Could you check a few things on this model? Use its own coordinates, in mm. Round coordinates to 2 decimals unless told otherwise and drop trailing zeros. Write each loop counter-clockwise with the first axis right and the second up, starting at its lowest first coordinate (ties: lowest second). Pieces come first, ordered by that corner, then holes. Notation, with made-up numbers: (75, -17) - (82, -17) arc R15 ccw to (82, 11) - close; hole circle Ø10 at (-33.5, 74). An arc over 180 degrees is marked (long way). Write each question's results on one line, items separated by ' | '. Start each with the question number.
(1) For P1, Ø2, axis at y = 44.5, z = -50, coming from the -X side; P2, Ø9, axis at y = 200, z = -15, coming from the -X side, each with a flat end and sliding along its axis, tell me the tip position at first contact or that it passes through.
(2) Please list where these lines run through material, in increasing order: line 1 (Z direction, x = 1.2, y = 200); line 2 (Z direction, x = 1.3, y = 44.5); line 3 (Y direction, x = 1.2, z = -87). Write a range as [from, to].
(3) Imagine slicing it at A-A on z = -43. Write out the boundary of the cut face in (x, y).
(4) Thinking about a two-plate mould opening in Z: for faces 1 (the flat face through (2, 133, -49)), 2 (the cylindrical face through (1, 218, -1)), 3 (the cylindrical face through (0.986, 200.759, -88.417)), 4 (the cylindrical face through (0.99, 196.66, -13.95)), which applies, +Z half, -Z half, draft (parallel to the pull), parting line (faces both ways), or undercut?
(5) Imagine slicing it at C-C on y = 200. Write out the boundary of the cut face in (x, z), then the cut area to 3 significant figures.
(6) Imagine slicing it at B-B on x = 0.4. Write out the boundary of the cut face in (y, z).
(7) Imagine slicing it at D-D on z = -15. Write out the boundary of the cut face in (x, y), then the cut area to 3 significant figures.
```python
from build123d import *

# Parameters (mm, degrees)
SKETCH_1_W          = 2
SKETCH_1_H          = 220
EXTRUDE_1_DEPTH     = 100
SKETCH_2_R          = 1.65
SKETCH_2_R_2        = 3.5
SKETCH_2_W          = 53
SKETCH_2_H          = 81
CUT_EXTRUDE_1_DEPTH = 10
FILLET_1_R          = 5


with BuildPart() as part:
    # 草图1 → 拉伸-薄壁1 (new body)
    with BuildSketch(Plane.XY):
        with Locations((1, 110)):
            Rectangle(SKETCH_1_W, SKETCH_1_H)
    extrude(amount=-EXTRUDE_1_DEPTH)

    # 草图2 → 切除-拉伸1 (cut)
    with BuildSketch(Plane.ZY):
        with Locations(Location((-50, 44.5, 0), (0, 0, 270))):
            Circle(SKETCH_2_R)
        with Locations(Location((-50, 134.5, 0), (0, 0, 270))):
            Circle(SKETCH_2_R)
        with Locations(Location((-15, 200, 0), (0, 0, 270))):
            Circle(SKETCH_2_R_2)
        with Locations(Location((-85, 200, 0), (0, 0, 270))):
            Circle(SKETCH_2_R_2)
        with Locations((-50, 89.5)):
            Rectangle(SKETCH_2_W, SKETCH_2_H)
        with BuildLine():
            Line((-11.5, 22.5), (-11.5, 17.5))
            ThreePointArc((-11.5, 17.5), (-15, 14), (-18.5, 17.5))
            Line((-18.5, 17.5), (-18.5, 22.5))
            ThreePointArc((-18.5, 22.5), (-15, 26), (-11.5, 22.5))
        make_face()
        with BuildLine():
            Line((-81.5, 22.5), (-81.5, 17.5))
            ThreePointArc((-81.5, 17.5), (-85, 14), (-88.5, 17.5))
            Line((-88.5, 17.5), (-88.5, 22.5))
            ThreePointArc((-88.5, 22.5), (-85, 26), (-81.5, 22.5))
        make_face()
    extrude(amount=-CUT_EXTRUDE_1_DEPTH, mode=Mode.SUBTRACT)

    # 圆角1
    fillet_1_edges = [part.edges().sort_by_distance(p)[0] for p in [
        (1, 220, -100),
        (1, 220, 0),
        (1, 0, 0),
        (1, 0, -100),
    ]]
    fillet(fillet_1_edges, radius=FILLET_1_R)


solid = part.part
```
Response:
1) P1: through | P2: x = 0
2) line 1: [-100, -88.5], [-81.5, -18.5], [-11.5, 0] | line 2: [-100, -51.65], [-48.35, 0] | line 3: [0, 14.63], [25.37, 197.13], [202.87, 220]
3) outline: (0, 0) - (2, 0) - (2, 49) - (0, 49) - close; (0, 130) - (2, 130) - (2, 220) - (0, 220) - close
4) face 1: draft | face 2: +Z half | face 3: undercut | face 4: undercut
5) outline: (0, -100) - (2, -100) - (2, -88.5) - (0, -88.5) - close; (0, -81.5) - (2, -81.5) - (2, -18.5) - (0, -18.5) - close; (0, -11.5) - (2, -11.5) - (2, 0) - (0, 0) - close | area: 172 mm²
6) outline: (0, -95) arc R5 ccw to (5, -100) - (215, -100) arc R5 ccw to (220, -95) - (220, -5) arc R5 ccw to (215, 0) - (5, 0) arc R5 ccw to (0, -5) - close; hole (17.5, -88.5) - (22.5, -88.5) arc R3.5 ccw to (22.5, -81.5) - (17.5, -81.5) arc R3.5 ccw to start; hole (17.5, -18.5) - (22.5, -18.5) arc R3.5 ccw to (22.5, -11.5) - (17.5, -11.5) arc R3.5 ccw to start; hole circle Ø3.3 at (44.5, -50); hole (49, -76.5) - (130, -76.5) - (130, -23.5) - (49, -23.5) - close; hole circle Ø3.3 at (134.5, -50); hole circle Ø7 at (200, -85); hole circle Ø7 at (200, -15)
7) outline: (0, 0) - (2, 0) - (2, 14) - (0, 14) - close; (0, 26) - (2, 26) - (2, 196.5) - (0, 196.5) - close; (0, 203.5) - (2, 203.5) - (2, 220) - (0, 220) - close | area: 402 mm²
